Check sheet for the modelled part. Datum: model origin and axes. Units: mm. A direction names the side the tool comes from. Round coordinates to 2 decimals unless told otherwise and drop trailing zeros. Loops run counter-clockwise (first coordinate to the right, second up) from the corner with the lowest first, then second, coordinate; pieces in that order, holes last. Notation, with made-up numbers: (-17.75, 35) -> (38.25, 35) arc R23 ccw to (38.25, 61) -> close; hole circle Ø3 at (19.5, 1). An arc over 180 degrees is marked (long way). Return JSON: item names as keys, results as strings.
from build123d import *

# Parameters (mm, degrees)
SKETCH3_OUTSIDE_W                       = 58.574
SKETCH3_OUTSIDE_H                       = 58.574
SKETCH3_OUTSIDE_W_2                     = 32
SKETCH3_OUTSIDE_H_2                     = 50
CUT_EXTRUDE1_DEPTH                      = 33.388269481
CBORE_FOR_M3_HEX_HEAD_BOLT1_D           = 3.5
CBORE_FOR_M3_HEX_HEAD_BOLT1_CBORE_D     = 6
CBORE_FOR_M3_HEX_HEAD_BOLT1_CBORE_DEPTH = 3.5


with BuildPart() as part:
    # Sketch1 → Revolve1 (revolve)
    with BuildSketch(Plane.XY, mode=Mode.PRIVATE) as revolve1_sk:
        Polygon((0, 9), (0, 22), (6, 22), (6, 14), (9, 14), (9, 12.5), (8, 12.5), (8, 9), align=None)
    revolve(revolve1_sk.sketch.rotate(Axis((0, 0, 0), (1, 0, 0)), 90), axis=Axis((0, 0, 0), (1, 0, 0)))

    # Sketch3 outside → Cut-Extrude1 (cut, through all)
    with BuildSketch(Plane.ZY):
        Rectangle(SKETCH3_OUTSIDE_W, SKETCH3_OUTSIDE_H)
        Rectangle(SKETCH3_OUTSIDE_W_2, SKETCH3_OUTSIDE_H_2, mode=Mode.SUBTRACT)
    extrude(amount=-CUT_EXTRUDE1_DEPTH, mode=Mode.SUBTRACT)

    # CBORE for M3 Hex Head Bolt1 (through all)
    with Locations(Plane.ZY):
        with Locations((0, 18), (0, -18)):
            CounterBoreHole(CBORE_FOR_M3_HEX_HEAD_BOLT1_D / 2, CBORE_FOR_M3_HEX_HEAD_BOLT1_CBORE_D / 2, CBORE_FOR_M3_HEX_HEAD_BOLT1_CBORE_DEPTH)


solid = part.part
Q1. Draft check along Y on faces 1 (the cylindrical face through (3, -22, 0)), 2 (the cylindrical face through (1.73, -20.93, -0.65)), 3 (the cylindrical face through (7.5, 12.4, 6.5)). Enter one of: released by +Y, released by -Y, zero draft, split by the parting line, or undercut.
Results list:
{"face 1": "released by -Y", "face 2": "undercut", "face 3": "split by the parting line"}
Q2. Tool access check on faces 4 (the flat face through (3.5, 16, 0)), 5 (the cylindrical face through (8.493, -3.755, 11.923)), 6 (the cylindrical face through (4.768, -16.265, 0.228)). Record the directions out of +Z, -Z, +X, -X, +Y, -Y that give a thin tool (end or side, any length) a straight path to the whole face; none if there is none.
Results list:
{"face 4": "-X", "face 5": "+X", "face 6": "+X, -X"}
Q3. Section check D-D (x = 6.5). Record the boundary of the cut face in (y, z).
Results list:
{"outline": "circle Ø28 at (0, 0); hole circle Ø18 at (0, 0)"}
Q4. Material ranges on line 1 (Y direction, x = 2.1, z = 0); line 2 (Y direction, x = 4.8, z = 0); line 3 (Y direction, x = 8.6, z = 0), recorded low to high.
Results list:
{"line 1": "-22 to -21, -15 to -9, 9 to 15, 21 to 22", "line 2": "-22 to -19.75, -16.25 to -9, 9 to 16.25, 19.75 to 22", "line 3": "-14 to -12.5, 12.5 to 14"}
Q5. Section check C-C (y = -18). Record the boundary of the cut face in (x, z).
Results list:
{"outline": "(0, -12.65) -> (6, -12.65) -> (6, -1.75) -> (3.5, -1.75) -> (3.5, -3) -> (0, -3) -> close; (0, 3) -> (3.5, 3) -> (3.5, 1.75) -> (6, 1.75) -> (6, 12.65) -> (0, 12.65) -> close"}
Q6. Section check A-A (z = 0). Count the separate pieces of the cut face and the enclosed holes in it, then the cut area to 4 significant figures.
Results list:
{"separate pieces": "4", "enclosed holes": "0", "area": "119.5 mm^2"}
Q7. Go/stop test with flat-tipped pins: pin 1 (2 mm diameter, centred on x = 8, z = 1.5, fed in from -Y); pin 2 (5 mm diameter, centred on y = -18, z = 0, fed in from -X); pin 3 (3 mm diameter, centred on y = 4, z = -8.5, fed in from +X). Record where each tip stops, or that it passes through.
Results list:
{"pin 1": "y = -13.99", "pin 2": "x = 3.5", "pin 3": "x = 8"}
Q8. Section check B-B (x = 4.5). Record the boundary of the cut face in (y, z), then the cut area to 3 significant figures.
Results list:
{"outline": "(-15.1, -16) -> (15.1, -16) arc R22 ccw to (15.1, 16) -> (-15.1, 16) arc R22 ccw to start; hole circle Ø3.5 at (-18, 0); hole circle Ø18 at (0, 0); hole circle Ø3.5 at (18, 0)", "area": "998 mm^2"}
